Geometry: see drawing. Coordinates: mm, zero at the bounding-box minimum. Coordinates: 2 decimals unless noted, no trailing zeros. Write each loop counter-clockwise with the first axis right and the second up, starting at its lowest first coordinate (ties: lowest second). Pieces come first, ordered by that corner, then holes. Notation, with made-up numbers: (3, -28.5) -> (53, -28.5) arc R22 cw to (53, -13.5) -> close; hole circle Ø3 at (67, -32). An arc over 180 degrees is marked (long way). Use one line per item in the form item = value. Start each with the question number.
(1) Cut plane C-C on z = 4.6. Return the cut outline in (x, y), plus the area to 3 significant figures.
(2) Cut plane A-A on x = 67. Return the cut outline in (y, z), plus the area to 3 significant figures.
(3) First-contact query: pin 1 (5 mm diameter, centred on x = 65, y = 8.5, fed in from -Z). Flat tip, straight axial feed; report the tip coordinate or a pass-through.
(4) Ray query, line 1 along Y through (x, z) = (10, 1.45); line 2 along Y through (x, z) = (8, 4.5); line 3 along X through (y, z) = (7, 2.65). Return the intervals inside material, ascending.
(5) Cut plane B-B on y = 64.5. Return the cut outline in (x, z).
(6) Pull-direction query (Y, two-part tool) for the marked faces 1, 2 and 3; classes: released by +Y, released by -Y, zero draft, split by the parting line, or undercut.
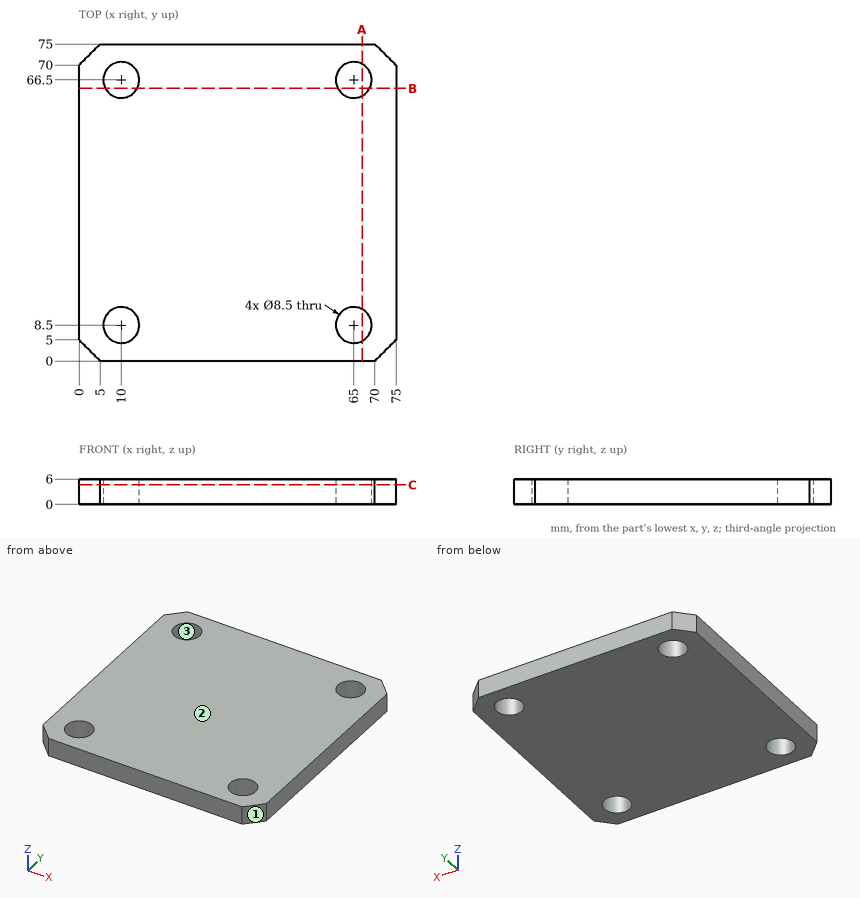
Values:
q1.outline = (0, 5) -> (5, 0) -> (70, 0) -> (75, 5) -> (75, 70) -> (70, 75) -> (5, 75) -> (0, 70) -> close; hole circle Ø8.5 at (10, 8.5); hole circle Ø8.5 at (10, 66.5); hole circle Ø8.5 at (65, 8.5); hole circle Ø8.5 at (65, 66.5)
q1.area = 5,350 mm2
q2.outline = (0, 0) -> (4.75, 0) -> (4.75, 6) -> (0, 6) -> close; (12.25, 0) -> (62.75, 0) -> (62.75, 6) -> (12.25, 6) -> close; (70.25, 0) -> (75, 0) -> (75, 6) -> (70.25, 6) -> close
q2.area = 360 mm2
q3.pin_1 = through
q4.line_1 = 0 to 4.25, 12.75 to 62.25, 70.75 to 75
q4.line_2 = 0 to 4.75, 12.25 to 62.75, 70.25 to 75
q4.line_3 = 0 to 6.02, 13.98 to 61.02, 68.98 to 75
q5.outline = (0, 0) -> (6.25, 0) -> (6.25, 6) -> (0, 6) -> close; (13.75, 0) -> (61.25, 0) -> (61.25, 6) -> (13.75, 6) -> close; (68.75, 0) -> (75, 0) -> (75, 6) -> (68.75, 6) -> close
q6.face_1 = released by -Y
q6.face_2 = zero draft
q6.face_3 = undercut
